Verification items for the finished model (mm, model axes). A direction names the side the tool comes from. Round coordinates to 2 decimals unless told otherwise and drop trailing zeros. Order: outer loops, then holes, each group sorted by start corner. A loop starts at its lowest first (then second) coordinate and runs counter-clockwise, first axis right, second up. Notation, with made-up numbers: (-7.75, -27.75) -> (-1.75, -27.75) arc R22 cw to (-1.75, -9.75) -> close; hole circle Ø4 at (-16.75, -24). An arc over 180 degrees is marked (long way). Return JSON: item names as keys, results as strings. Group by question number.
Item 1: Access from +Z, -Z, +X, -X, +Y, -Y to the whole of each face (thin tool, end or side, straight path). Record for faces 1 (the flat face through (-37, -1, 10)), 2 (the cylindrical face through (-35.494, 0.264, 15.14)), 3 (the flat face through (-30, 28, 10)).
Item 2: Depth check by flat-ended pin: pin 1 Ø7.5 at (x, y) = (-31.5, -25.5) entering from +Z; pin 2 Ø1.5 at (x, z) = (-25, 12.5) entering from -Y; pin 3 Ø4.5 at (x, z) = (-28.5, 19.5) entering from +Y; pin 4 Ø3.5 at (x, y) = (-26.5, 30) entering from +Z. Enter the tip coordinate at first touch or a pass-through.
Item 3: Sectioned sample at A-A on z = 6. Record the cut outline in (x, y).
Item 4: Draft check along Y on faces 4 (the flat face through (-30, -27, 10)), 5 (the flat face through (-30, 17.5, 18)), 6 (the cylindrical face through (-24.59, 29.21, 5.07)), 7 (the flat face through (-30, -17.5, 18)). Enter one of: pulls with the +Y half, pulls with the -Y half, needs draft (parallel to the pull), parting line crosses it, or undercut.
Item 5: Scan lines: probe 1 along Y at (x, z) = (-26.5, 2); probe 2 along Y at (x, z) = (-29.5, 10.25); probe 3 along Z at (x, y) = (-26, -23). Record each from-to range of solid material in increasing order. Write a range as from..to.
Item 6: Sectioned sample at B-B on y = 30. Record the cut outline in (x, z).
Item 7: Sectioned sample at C-C on x = -26.75. Record the cut outline in (y, z), plus the area to 3 significant figures.
Item 8: Sectioned sample at D-D on z = 2. Record the cut outline in (x, y), plus the area to 3 significant figures.
```python
from build123d import *

# Parameters (mm, degrees)
SKETCH1_W           = 15
SKETCH1_H           = 75
BOSS_EXTRUDE1_DEPTH = 25
SKETCH2_R           = 2.067
CUT_EXTRUDE1_DEPTH  = 25
SKETCH3_W           = 15
SKETCH3_H           = 20
CUT_EXTRUDE2_DEPTH  = 15
SKETCH4_R           = 6
CUT_EXTRUDE3_DEPTH  = 20


with BuildPart() as part:
    # Sketch1 → Boss-Extrude1 (new body)
    with BuildSketch(Plane.XY):
        with Locations((-29.5, 0)):
            Rectangle(SKETCH1_W, SKETCH1_H)
    extrude(amount=BOSS_EXTRUDE1_DEPTH)

    # Sketch2 → Cut-Extrude1 (cut)
    with BuildSketch(Plane.XY.offset(25)):
        with Locations((-26.5, 30)):
            Circle(SKETCH2_R)
        with Locations((-26.5, -30)):
            Circle(SKETCH2_R)
    extrude(amount=-CUT_EXTRUDE1_DEPTH, mode=Mode.SUBTRACT)

    # Sketch3 → Cut-Extrude2 (cut)
    with BuildSketch(Plane.XY.offset(25)):
        with Locations((-29.5, 27.5)):
            Rectangle(SKETCH3_W, SKETCH3_H)
        with Locations((-29.5, -27.5)):
            Rectangle(SKETCH3_W, SKETCH3_H)
    extrude(amount=-CUT_EXTRUDE2_DEPTH, mode=Mode.SUBTRACT)

    # Sketch4 → Cut-Extrude3 (cut)
    with BuildSketch(Plane.XY.offset(25)):
        with Locations((-29.5, 0)):
            Circle(SKETCH4_R)
    extrude(amount=-CUT_EXTRUDE3_DEPTH, mode=Mode.SUBTRACT)


solid = part.part
```
Recorded:
{
 "1": {"face 1": "+Z, -Z, -X, +Y, -Y", "face 2": "+Z", "face 3": "+Z, +X, -X, +Y"},
 "2": {"pin 1": "z = 10", "pin 2": "y = -17.5", "pin 3": "y = 17.5", "pin 4": "through"},
 "3": {"outline": "(-37, -37.5) -> (-22, -37.5) -> (-22, 37.5) -> (-37, 37.5) -> close; hole circle Ø12 at (-29.5, 0); hole circle Ø4.13 at (-26.5, -30); hole circle Ø4.13 at (-26.5, 30)"},
 "4": {"face 4": "needs draft", "face 5": "pulls with the +Y half", "face 6": "undercut", "face 7": "pulls with the -Y half"},
 "5": {"probe 1": "-37.5..-32.07, -27.93..27.93, 32.07..37.5", "probe 2": "-17.5..-6, 6..17.5", "probe 3": "0..10"},
 "6": {"outline": "(-37, 0) -> (-28.57, 0) -> (-28.57, 10) -> (-37, 10) -> close; (-24.43, 0) -> (-22, 0) -> (-22, 10) -> (-24.43, 10) -> close"},
 "7": {"outline": "(-37.5, 0) -> (-32.05, 0) -> (-32.05, 10) -> (-37.5, 10) -> close; (-27.95, 0) -> (27.95, 0) -> (27.95, 10) -> (17.5, 10) -> (17.5, 25) -> (5.33, 25) -> (5.33, 5) -> (-5.33, 5) -> (-5.33, 25) -> (-17.5, 25) -> (-17.5, 10) -> (-27.95, 10) -> close; (32.05, 0) -> (37.5, 0) -> (37.5, 10) -> (32.05, 10) -> close", "area": "980 mm²"},
 "8": {"outline": "(-37, -37.5) -> (-22, -37.5) -> (-22, 37.5) -> (-37, 37.5) -> close; hole circle Ø4.13 at (-26.5, -30); hole circle Ø4.13 at (-26.5, 30)", "area": "1,100 mm²"}
}
